from build123d import *

# Parameters (mm, degrees)
SKETCH_4_OUTSIDE_W       = 260.734
SKETCH_4_OUTSIDE_H       = 260.734
SKETCH_4_OUTSIDE_R       = 22.5
CUT_EXTRUDE_2_DEPTH      = 2.2
HOLE_WIZARD_M10_1_D      = 8.5
PATTERN_CIRCULAR_1_COUNT = 4
CUT_EXTRUDE_5_DEPTH      = 154.242815166
HOLE_WIZARD_M10_2_D      = 8.5
HOLE_WIZARD_M10_2_DEPTH  = 60
HOLE_WIZARD_M10_2_TIP    = 2.553657631


with BuildPart() as part:
    # 草图1 → 旋转1 (revolve)
    with BuildSketch(Plane(origin=(0, 0, 0), x_dir=(1, 0, 0), z_dir=(0, 1, 0))):
        Polygon((0, 0), (-100, 0), (-100, 20), (-26.5, 20), (-26.5, 49.02), (-25, 49.02), (-25, 79.02), (0, 79.02), align=None)
    revolve(axis=Axis((0, 0, 0), (0, 0, 1)))

    # 草图4 outside → 切除-拉伸2 (cut)
    with BuildSketch(Plane(origin=(0, 0, -74.52), x_dir=(-1, 0, 0), z_dir=(0, 0, -1))):
        Rectangle(SKETCH_4_OUTSIDE_W, SKETCH_4_OUTSIDE_H)
        Circle(SKETCH_4_OUTSIDE_R, mode=Mode.SUBTRACT)
    extrude(amount=CUT_EXTRUDE_2_DEPTH, mode=Mode.SUBTRACT)

    # M10 螺纹孔1 (through all)
    with Locations(Plane(origin=(0, 0, -20), x_dir=(-1, 0, 0), z_dir=(0, 0, -1))):
        with Locations((0, -80)):
            hole_wizard_m10_1 = Hole(HOLE_WIZARD_M10_1_D / 2)

    # 阵列(圆周)1: M10 螺纹孔1 ×4 about axis
    pattern_circular_1_axis = Axis((0, 0, 0), (0, 0, 1))
    for i in range(1, PATTERN_CIRCULAR_1_COUNT):
        add(hole_wizard_m10_1.rotate(pattern_circular_1_axis, i * 360 / PATTERN_CIRCULAR_1_COUNT), mode=Mode.SUBTRACT)

    # 草图10 → 切除-拉伸5 (cut, through all)
    with BuildSketch(Plane(origin=(0, 0, -20), x_dir=(-1, 0, 0), z_dir=(0, 0, -1))):
        Polygon((106.066017178, 21.213203436), (21.213203436, 106.066017178), (56.786089274, 141.638903017), (141.638903017, 56.786089274), align=None)
    extrude(amount=-CUT_EXTRUDE_5_DEPTH, mode=Mode.SUBTRACT)

    # M10 螺纹孔2
    with Locations(Plane(origin=(-63.639610307, 63.639610307, 0), x_dir=(0.7071067811865476, 0.7071067811865475, 0), z_dir=(-0.7071067811865475, 0.7071067811865476, 0))):
        with Locations((0, 12)):
            Hole(HOLE_WIZARD_M10_2_D / 2, depth=HOLE_WIZARD_M10_2_DEPTH)
            with Locations((0, 0, -(HOLE_WIZARD_M10_2_DEPTH + HOLE_WIZARD_M10_2_TIP / 2))):  # 118° drill point
                Cone(0, HOLE_WIZARD_M10_2_D / 2, HOLE_WIZARD_M10_2_TIP, mode=Mode.SUBTRACT)


solid = part.part
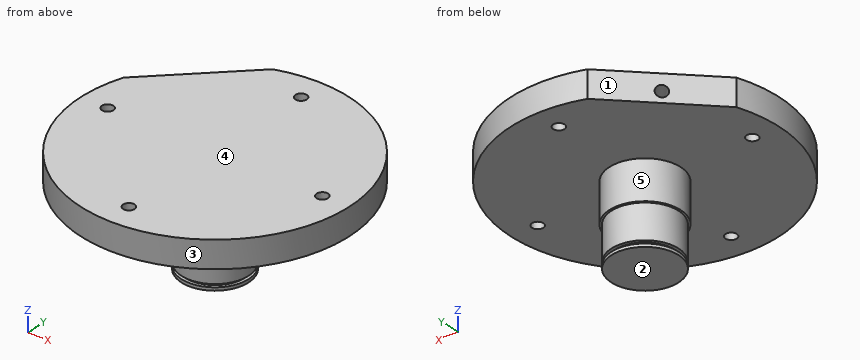
Source: CAD feature listing. Evaluate the final solid. Frame: model axes, mm. Face numbers are marked on the shaded views. A direction names the side the tool comes from. Round coordinates to 2 decimals unless told otherwise and drop trailing zeros. Loops run counter-clockwise (first coordinate to the right, second up) from the corner with the lowest first, then second, coordinate; pieces in that order, holes last.
Q1. Section C-C, the plane x = -80. Return loops of the section in (y, z).
Q2. First-contact query: P1, Ø1.5, axis at x = -45, y = 67.5, coming from the -Z side; P2, Ø12, axis at y = -3, z = -66.5, coming from the -X side; P3, Ø3, axis at x = 21, z = -66.5, coming from the -Y side. Flat tips, straight axial feed; report the tip coordinate or a pass-through.
Q3. Section A-A, the plane x = 0. Return loops of the section in (y, z).
Q4. Access query for the marked faces 4 and 5. Directions: +Z, -Z, +X, -X, +Y, -Y. A direction counts if a zero-diameter tool reaches every point of the face in a straight line with its end or side. Return the directions, or none.
Q5. Mould query, pull axis Y, two halves, no side actions, for the marked faces 1, 2 and 3. Classes: pulls with the +Y half, pulls with the -Y half, needs draft (parallel to the pull), parting line crosses it, or undercut.
Q6. Section D-D, the plane y = 80. Return loops of the section in (x, z).
Q7. Ray query, line 1 (Y direction, x = 0, z = -6.75); line 2 (Z direction, x = -62, y = 53). Return the intervals inside material, ascending.
Solutions:
1. outline: (-60, -20) - (-4.25, -20) - (-4.25, 0) - (-60, 0) - close; (4.25, -20) - (47.28, -20) - (47.28, 0) - (4.25, 0) - close
2. P1: stops at z = -20
2. P2: stops at x = -25
2. P3: stops at y = -15.64
3. outline: (-100, -20) - (-84.25, -20) - (-84.25, 0) - (-100, 0) - close; (-75.75, -20) - (-26.5, -20) - (-26.5, -49.02) - (-25, -49.02) - (-25, -74.52) - (-22.5, -74.52) - (-22.5, -76.72) - (-25, -76.72) - (-25, -79.02) - (25, -79.02) - (25, -76.72) - (22.5, -76.72) - (22.5, -74.52) - (25, -74.52) - (25, -49.02) - (26.5, -49.02) - (26.5, -20) - (75.75, -20) - (75.75, 0) - (-75.75, 0) - close; (84.25, -20) - (100, -20) - (100, 0) - (84.25, 0) - close
4. face 4: +Z, +X, -X, +Y, -Y
4. face 5: -Z
5. face 1: pulls with the +Y half
5. face 2: needs draft
5. face 3: parting line crosses it
6. outline: (-47.28, -20) - (-4.25, -20) - (-4.25, 0) - (-47.28, 0) - close; (4.25, -20) - (60, -20) - (60, 0) - (4.25, 0) - close
7. line 1: y = -100 to -84.25, -75.75 to 75.75, 84.25 to 100
7. line 2: z = -20 to 0
